Could you check a few things on this model? Use its own coordinates, in mm. A direction names the side the tool comes from. Coordinates: 2 decimals unless noted, no trailing zeros. Write each loop counter-clockwise with the first axis right and the second up, starting at its lowest first coordinate (ties: lowest second). Pieces come first, ordered by that corner, then holes.
Item 1: I want a section at D-D on y = 23.75. Please give me the cut outline in (x, z).
Item 2: I want a section at A-A on z = 6. Please give me the cut outline in (x, y).
Item 3: For P1, Ø5, axis at y = 20.5, z = 1.5, coming from the +X side; P2, Ø6, axis at x = 32, z = 7, coming from the +Y side, each with a flat end and sliding along its axis, tell me the tip position at first contact or that it passes through.
Item 4: Which directions (+Z, -Z, +X, -X, +Y, -Y) give clear straight access to the entire face, cutting with the end or side of a thin tool? Please do faces 5 (the cylindrical face through (5.25, 9.63, 5.94)), 6 (the cylindrical face through (1, 13, 2)), 7 (the flat face through (20, 19, 3)).
Item 5: I want a section at C-C on x = 25. Please give me the cut outline in (y, z), then the cut area to 4 significant figures.
Item 6: I want a section at B-B on y = 2.5. Please give me the cut outline in (x, z).
Item 7: Thinking about a two-plate mould opening in X: for faces 1 (the cylindrical face through (34.75, 9.63, 6.06)), 2 (the flat face through (40, 12, 8)), 3 (the cylindrical face through (3, 22, 6)), 4 (the flat face through (0, 12, 8)), which applies, +X half, -X half, draft (parallel to the pull), parting line (faces both ways), or undercut?
Item 8: If I drill on probe 1 along Z at (x, y) = (32, 18.75); probe 2 along X at (y, z) = (22.5, 1.75), over which ranges is the centre line in solid material (lowest first)?
from build123d import *

# Parameters (mm, degrees)
SKETCH_1_W          = 40
SKETCH_1_H          = 25
EXTRUDE_1_DEPTH     = 12
CUT_EXTRUDE_1_DEPTH = 6
CUT_EXTRUDE_2_DEPTH = 19
FILLET_1_R          = 5


with BuildPart() as part:
    # 草图1 → 凸台-拉伸1 (new body)
    with BuildSketch(Plane.XY):
        with Locations((20, 12.5)):
            Rectangle(SKETCH_1_W, SKETCH_1_H)
    extrude(amount=EXTRUDE_1_DEPTH)

    # 草图4 → 切除-拉伸1 (cut)
    with BuildSketch(Plane(origin=(0, 25, 0), x_dir=(1, 0, 0), z_dir=(0, 1, 0))):
        with BuildLine():
            Line((8, -1), (32, -1))
            ThreePointArc((32, -1), (37, -6), (32, -11))
            Line((32, -11), (8, -11))
            ThreePointArc((8, -11), (3, -6), (8, -1))
        make_face()
    extrude(amount=-CUT_EXTRUDE_1_DEPTH, mode=Mode.SUBTRACT)

    # 草图5 → 切除-拉伸2 (cut)
    with BuildSketch(Plane(origin=(0, 19, 0), x_dir=(1, 0, 0), z_dir=(0, 1, 0))):
        with BuildLine():
            Line((8, -8.75), (32, -8.75))
            ThreePointArc((32, -8.75), (34.75, -6), (32, -3.25))
            Line((32, -3.25), (8, -3.25))
            ThreePointArc((8, -3.25), (5.25, -6), (8, -8.75))
        make_face()
    extrude(amount=-CUT_EXTRUDE_2_DEPTH, mode=Mode.SUBTRACT)

    # 圆角1
    fillet_1_edges = [part.edges().sort_by_distance(p)[0] for p in [
        (40, 12.5, 0),
        (0, 12.5, 0),
    ]]
    fillet(fillet_1_edges, radius=FILLET_1_R)


solid = part.part
Response values:
1. outline: (0, 5) arc R5 ccw to (5, 0) - (35, 0) arc R5 ccw to (40, 5) - (40, 12) - (0, 12) - close; hole (8, 1) - (32, 1) arc R5 ccw to (32, 11) - (8, 11) arc R5 ccw to start
2. outline: (0, 0) - (5.25, 0) - (5.25, 19) - (3, 19) - (3, 25) - (0, 25) - close; (34.75, 0) - (40, 0) - (40, 25) - (37, 25) - (37, 19) - (34.75, 19) - close
3. P1: stops at x = 39.9
3. P2: stops at y = 19
4. face 5: +Y, -Y
4. face 6: -Z, -X, +Y, -Y
4. face 7: +Y
5. outline: (0, 0) - (25, 0) - (25, 1) - (19, 1) - (19, 3.25) - (0, 3.25) - close; (0, 8.75) - (19, 8.75) - (19, 11) - (25, 11) - (25, 12) - (0, 12) - close
5. area: 135.5 mm2
6. outline: (0, 5) arc R5 ccw to (5, 0) - (35, 0) arc R5 ccw to (40, 5) - (40, 12) - (0, 12) - close; hole (8, 3.25) - (32, 3.25) arc R2.75 ccw to (32, 8.75) - (8, 8.75) arc R2.75 ccw to start
7. face 1: undercut
7. face 2: +X half
7. face 3: undercut
7. face 4: -X half
8. probe 1: z = 0 to 3.25, 8.75 to 12
8. probe 2: x = 1.2 to 5.37, 34.63 to 38.8
